Design review of the part built by this model. Coordinates are the model's own, in mm. Face numbers are marked on the shaded views. Round coordinates to 2 decimals unless told otherwise and drop trailing zeros. Loops run counter-clockwise (first coordinate to the right, second up) from the corner with the lowest first, then second, coordinate; pieces in that order, holes last. Notation, with made-up numbers: M 83.25,41 L 102.25,41 A13 cw 102.25,57 Z; hole C -13,-37 d1. An arc over 180 degrees is marked long. Use a Markdown table: item, result.
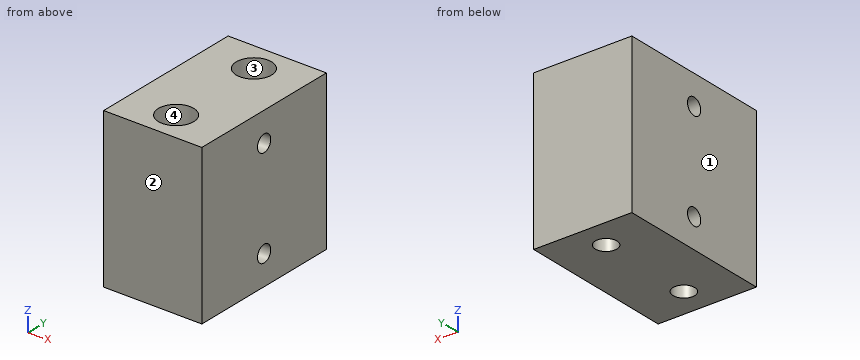
from build123d import *

# Parameters (mm, degrees)
SKETCH_1_W                = 80
SKETCH_1_H                = 80
EXTRUDE_1_DEPTH           = 50
HOLE_WIZARD_1_D           = 11
HOLE_WIZARD_1_CBORE_D     = 18
HOLE_WIZARD_1_CBORE_DEPTH = 30
HOLE_WIZARD_M10_1_D       = 8.5


with BuildPart() as part:
    # 草图1 → 凸台-拉伸1 (new body)
    with BuildSketch(Plane(origin=(0, 0, 0), x_dir=(0, 0, -1), z_dir=(1, 0, 0))):
        Rectangle(SKETCH_1_W, SKETCH_1_H)
    extrude(amount=EXTRUDE_1_DEPTH)

    # 打孔尺寸(%根据)内六角圆柱头螺钉的类型1 (through all)
    with Locations(Plane.XY.offset(40)):
        with Locations((25, 25), (25, -25)):
            CounterBoreHole(HOLE_WIZARD_1_D / 2, HOLE_WIZARD_1_CBORE_D / 2, HOLE_WIZARD_1_CBORE_DEPTH)

    # M10 螺纹孔1 (through all)
    with Locations(Plane(origin=(50, 0, 0), x_dir=(0, 0, -1), z_dir=(1, 0, 0))):
        with Locations((25, 0), (-25, 0)):
            Hole(HOLE_WIZARD_M10_1_D / 2)


solid = part.part
1. Take a section at C-C on y = 0. Give the boundary of the cut face in (x, z).
Check values:
| item | result |
|---|---|
| outline | M 0,-40 L 50,-40 L 50,-29.25 L 0,-29.25 Z; M 0,-20.75 L 50,-20.75 L 50,20.75 L 0,20.75 Z; M 0,29.25 L 50,29.25 L 50,40 L 0,40 Z |
2. Take a section at D-D on y = 25. Give the boundary of the cut face in (x, z).
Check values:
| item | result |
|---|---|
| outline | M 0,-40 L 19.5,-40 L 19.5,10 L 16,10 L 16,40 L 0,40 Z; M 30.5,-40 L 50,-40 L 50,40 L 34,40 L 34,10 L 30.5,10 Z |
3. The part is to be moulded in two halves that separate along X. For the marked faces 1, 2, 3 and 4, say which applies: pulls with the +X half, pulls with the -X half, needs draft (parallel to the pull), parting line crosses it, or undercut.
Check values:
| item | result |
|---|---|
| face 1 | pulls with the -X half |
| face 2 | needs draft |
| face 3 | undercut |
| face 4 | undercut |
4. Wall thickness on line 1 along Y through (x, z) = (25, 25); line 2 along Z through (x, y) = (34.5, -1); line 3 along Y through (x, z) = (14, -25): over which ranges is each line inside the solid? List them lowest first. Write a range as from..to.
Check values:
| item | result |
|---|---|
| line 1 | y = -40..-34, -16..-4.25, 4.25..16, 34..40 |
| line 2 | z = -40..-29.13, -20.87..20.87, 29.13..40 |
| line 3 | y = -40..-4.25, 4.25..40 |
5. Take a section at B-B on z = -5. Give the boundary of the cut face in (x, y), and give its area (3 significant figures).
Check values:
| item | result |
|---|---|
| outline | M 0,-40 L 50,-40 L 50,40 L 0,40 Z; hole C 25,-25 d11; hole C 25,25 d11 |
| area | 3,810 mm² |
6. Insertion check: pin 1 (10 mm diameter, centred on x = 25, y = 25, fed in from -Z); pin 2 (2 mm diameter, centred on x = 24, y = 29.5, fed in from +Z). Each pin has a flat end and moves straight along its axis. Give the tip position at first contact, or say it passes through.
Check values:
| item | result |
|---|---|
| pin 1 | passes through |
| pin 2 | stops at z = 10 |
7. Take a section at A-A on x = 25. Give the boundary of the cut face in (y, z).
Check values:
| item | result |
|---|---|
| outline | M -40,-40 L -30.5,-40 L -30.5,10 L -34,10 L -34,40 L -40,40 Z; M -19.5,-40 L 19.5,-40 L 19.5,10 L 16,10 L 16,40 L -16,40 L -16,10 L -19.5,10 Z; M 30.5,-40 L 40,-40 L 40,40 L 34,40 L 34,10 L 30.5,10 Z; hole C 0,-25 d8.5; hole C 0,25 d8.5 |
